Part model, mm, in its own coordinate system. Face numbers are marked on the shaded views. A direction names the side the tool comes from. Coordinates: 2 decimals unless noted, no trailing zeros. Order: outer loops, then holes, each group sorted by start corner. A loop starts at its lowest first (then second) coordinate and runs counter-clockwise, first axis right, second up. Notation, with made-up numbers: (52, -20) - (75, -20) arc R18 cw to (75, -15) - close; hole circle Ø2 at (61.5, 82). An arc over 180 degrees is marked (long way). Use a Markdown table: item, result. Add a question column.
1) Tool access for the marked faces 5, 6 and 7: list every direction of +Z, -Z, +X, -X, +Y, -Y with a clear straight run to the whole face (end or side of a thin tool).
2) Saw through at C-C on x = 7. List the corners of the cut face in (y, z) (3 decimals).
3) Drop flat-ended pins along their axis: P1, Ø3.5, axis at x = 1, z = -9.5, coming from the +Y side (3 decimals); P2, Ø6.5, axis at y = -47.77, z = 10, coming from the +X side (3 decimals); P3, Ø4, axis at y = -47.77, z = -10, coming from the +X side; P4, Ø1.5, axis at y = -0.5, z = -12.5, coming from the -X side (3 decimals). Give the stop position or say it passes through.
4) Saw through at A-A on z = -2.5. List the corners of the cut face in (x, y) (3 decimals), then the cut area to 3 significant figures.
5) Saw through at D-D on x = -1.5. List the corners of the cut face in (y, z) (3 decimals).
6) Two-plate mould, pull along Y, no slides. Class the marked faces 1, 2, 3 and 4: +Y half, -Y half, draft (parallel to the pull), parting line (faces both ways), or undercut.
7) Wall check: L1, parallel to Y at x = -4.9, z = 10 (3 decimals); L2, parallel to Y at x = -3.4, z = 10 (3 decimals); L3, parallel to X at y = -40, z = -15 (3 decimals). Give the ranges that are in metal, low to high. Write a range as [from, to].
8) Saw through at B-B on z = -10. List the corners of the cut face in (x, y) (3 decimals), then the cut area to 3 significant figures.
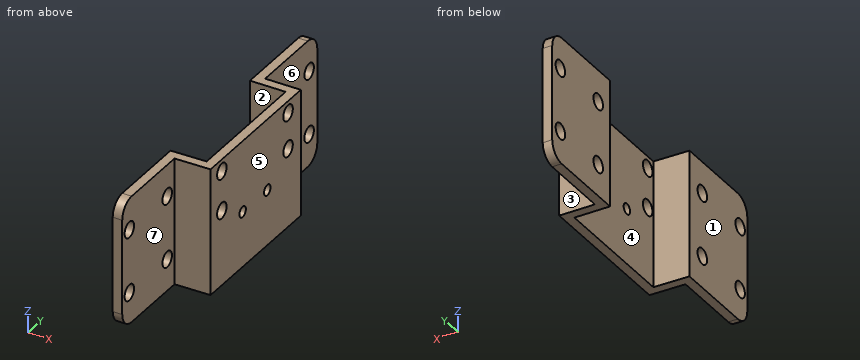
```python
from build123d import *

# Parameters (mm, degrees)
EXTRUDE_THIN1_DEPTH   = 20
FILLET1_R             = 5
SIZE_MM_DOWEL_HOLE1_D = 5
M4_TAPPED_HOLE1_D     = 3.4


with BuildPart() as part:
    # Sketch1 → Extrude-Thin1 (new, symmetric)
    with BuildSketch(Plane.XY):
        Polygon((-5.625, 51.525), (-5.625, 20.975), (5.625, 20.975), (5.625, -20.777349891), (-5.625, -20.974615696), (-5.625, -51.525), (-2.625, -51.525), (-2.625, -23.922472646), (8.625, -23.725206841), (8.625, 23.975), (-2.625, 23.975), (-2.625, 51.525), align=None)
    extrude(amount=EXTRUDE_THIN1_DEPTH, both=True)

    # Fillet1
    fillet1_edges = [part.edges().sort_by_distance(p)[0] for p in [
        (-4.125, 51.525, -20),
        (-4.125, -51.525, -20),
        (-4.125, 51.525, 20),
        (-4.125, -51.525, 20),
    ]]
    fillet(fillet1_edges, radius=FILLET1_R)

    # Size mm Dowel Hole1 (through all)
    with Locations(Plane(origin=(8.625, 0, 0), x_dir=(0, 0, -1), z_dir=(1, 0, 0))):
        with Locations((-3.75, -17.768125), (-16.25, -17.768125), (-4.858090708, 17.231875), (-16.25, 17.231875), (10, 47.231875), (10, 27.231875), (-10, 27.231875), (-10, 47.231875), (10, -47.768125), (10, -27.768125), (-10, -27.768125), (-10, -47.768125)):
            Hole(SIZE_MM_DOWEL_HOLE1_D / 2)

    # M4 Tapped Hole1 (through all)
    with Locations(Plane(origin=(8.625, 0, 0), x_dir=(0, 0, -1), z_dir=(1, 0, 0))):
        with Locations((2.5, -6.768125), (2.5, 6.231875)):
            Hole(M4_TAPPED_HOLE1_D / 2)


solid = part.part
```
Results are:
| question | item | result |
|---|---|---|
| 1 | face 5 | +Z, -Z, +X, +Y, -Y |
| 1 | face 6 | +Z, -Z, +X, +Y |
| 1 | face 7 | +Z, -Z, +X, -Y |
| 2 | outline | (-23.754, -20) - (23.975, -20) - (23.975, 20) - (-23.754, 20) - close; hole circle Ø5 at (-17.768, 3.75); hole circle Ø5 at (-17.768, 16.25); hole circle Ø3.4 at (-6.768, -2.5); hole circle Ø3.4 at (6.232, -2.5); hole circle Ø5 at (17.232, 4.858); hole circle Ø5 at (17.232, 16.25) |
| 3 | P1 | y = 23.975 |
| 3 | P2 | x = -2.625 |
| 3 | P3 | through |
| 3 | P4 | x = 5.625 |
| 4 | outline | (-5.625, -51.525) - (-2.625, -51.525) - (-2.625, -23.922) - (8.625, -23.725) - (8.625, -8.468) - (5.625, -8.468) - (5.625, -20.777) - (-5.625, -20.975) - close; (-5.625, 20.975) - (5.625, 20.975) - (5.625, 7.932) - (8.625, 7.932) - (8.625, 23.975) - (-2.625, 23.975) - (-2.625, 51.525) - (-5.625, 51.525) - close; (5.625, -5.068) - (8.625, -5.068) - (8.625, 4.532) - (5.625, 4.532) - close |
| 4 | area | 356 mm2 |
| 5 | outline | (-23.903, -20) - (-20.902, -20) - (-20.902, 20) - (-23.903, 20) - close; (20.975, -20) - (23.975, -20) - (23.975, 20) - (20.975, 20) - close |
| 6 | face 1 | draft |
| 6 | face 2 | undercut |
| 6 | face 3 | +Y half |
| 6 | face 4 | undercut |
| 7 | L1 | [-51.525, -50.268], [-45.268, -30.268], [-25.268, -20.962], [20.975, 24.732], [29.732, 44.732], [49.732, 51.525] |
| 7 | L2 | [-51.525, -50.268], [-45.268, -30.268], [-25.268, -20.936], [20.975, 24.732], [29.732, 44.732], [49.732, 51.525] |
| 7 | L3 | [-5.625, -2.625] |
| 8 | outline | (-5.625, -51.525) - (-2.625, -51.525) - (-2.625, -50.268) - (-5.625, -50.268) - close; (-5.625, -45.268) - (-2.625, -45.268) - (-2.625, -30.268) - (-5.625, -30.268) - close; (-5.625, -25.268) - (-2.625, -25.268) - (-2.625, -23.922) - (8.625, -23.725) - (8.625, 23.975) - (-2.625, 23.975) - (-2.625, 24.732) - (-5.625, 24.732) - (-5.625, 20.975) - (5.625, 20.975) - (5.625, -20.777) - (-5.625, -20.975) - close; (-5.625, 29.732) - (-2.625, 29.732) - (-2.625, 44.732) - (-5.625, 44.732) - close; (-5.625, 49.732) - (-2.625, 49.732) - (-2.625, 51.525) - (-5.625, 51.525) - close |
| 8 | area | 316 mm2 |
